```python
from build123d import *

# Parameters (mm, degrees)
SKETCH1_W           = 22
SKETCH1_H           = 8
BOSS_EXTRUDE1_DEPTH = 175
SKETCH2_R           = 2
CUT_EXTRUDE1_DEPTH  = 177.558772085


with BuildPart() as part:
    # Sketch1 → Boss-Extrude1 (new body)
    with BuildSketch(Plane.XY):
        with Locations((11, 4)):
            Rectangle(SKETCH1_W, SKETCH1_H)
    extrude(amount=BOSS_EXTRUDE1_DEPTH)

    # Sketch2 → Cut-Extrude1 (cut, through all)
    with BuildSketch(Plane(origin=(22, 0, 0), x_dir=(0, 0, -1), z_dir=(1, 0, 0))):
        with Locations((-4, 4)):
            Circle(SKETCH2_R)
        with Locations((-171, 4)):
            Circle(SKETCH2_R)
        with Locations((-29, 4)):
            Circle(SKETCH2_R)
    extrude(amount=-CUT_EXTRUDE1_DEPTH, mode=Mode.SUBTRACT)


solid = part.part
```
Work out the finished part from the listing and answer in its coordinate system (mm). Give positions to 0.01 mm unless a question says otherwise; leave off trailing zeros. Loops run counter-clockwise (first coordinate to the right, second up) from the corner with the lowest first, then second, coordinate; pieces in that order, holes last. Notation, with made-up numbers: M -10,7.5 L 39,7.5 A13 ccw 39,32.5 Z; hole C 30,54.5 d5. An arc over 180 degrees is marked long. One line per item, written item: value. Start each with the question number.
1. Find section A-A (y = 4). Give the vertices of the cut face in (x, z).
2. Find the intervals of material crossed by probe 1 along Y at (x, z) = (10.5, 171); probe 2 along Z at (x, y) = (9.75, 5); probe 3 along Z at (x, y) = (7.25, 5.75), in increasing order.
3. Find section C-C (x = 11). Give the vertices of the cut face in (y, z), and give its area (3 significant figures).
4. This flat-tipped pin is pushed along its axis until it touches: P1, Ø3, axis at y = 4, z = 29, coming from the -X side (3 decimals). Where does it stop, or does it pass through?
5. Determine the mould class of faces 1 (the face through (22, 4, 86)), 2 (the face through (11, 4, 173)), 3 (the face through (11, 4, 0)), 4 (the face through (11.154, 4.601, 27.092)) for opening direction Z: released by +Z, released by -Z, zero draft, split by the parting line, or undercut.
6. Find section B-B (z = 29). Give the vertices of the cut face in (x, y), and give its area (3 significant figures).
Reported:
1. outline: M 0,0 L 22,0 L 22,2 L 0,2 Z; M 0,6 L 22,6 L 22,27 L 0,27 Z; M 0,31 L 22,31 L 22,169 L 0,169 Z; M 0,173 L 22,173 L 22,175 L 0,175 Z
2. probe 1: y = 0 to 2, 6 to 8
2. probe 2: z = 0 to 2.27, 5.73 to 27.27, 30.73 to 169.27, 172.73 to 175
2. probe 3: z = 0 to 3.03, 4.97 to 28.03, 29.97 to 170.03, 171.97 to 175
3. outline: M 0,0 L 8,0 L 8,175 L 0,175 Z; hole C 4,4 d4; hole C 4,29 d4; hole C 4,171 d4
3. area: 1,360 mm²
4. P1: passes through
5. face 1: zero draft
5. face 2: undercut
5. face 3: released by -Z
5. face 4: undercut
6. outline: M 0,0 L 22,0 L 22,2 L 0,2 Z; M 0,6 L 22,6 L 22,8 L 0,8 Z
6. area: 88.0 mm²
